from build123d import *

# Parameters (mm, degrees)
SKETCH_1_R          = 30
SKETCH_1_R_2        = 17.5
EXTRUDE_1_DEPTH     = 17.5
SKETCH_2_R          = 21
CUT_EXTRUDE_1_DEPTH = 13
CHAMFER_1_SIZE      = 1


with BuildPart() as part:
    # 草图1 → 凸台-拉伸1 (new, symmetric)
    with BuildSketch(Plane.XY):
        Circle(SKETCH_1_R)
        Circle(SKETCH_1_R_2, mode=Mode.SUBTRACT)
    extrude(amount=EXTRUDE_1_DEPTH, both=True)

    # 草图2 → 切除-拉伸1 (cut)
    with BuildSketch(Plane.XY.offset(17.5)):
        Circle(SKETCH_2_R)
    cut_extrude_1 = extrude(amount=-CUT_EXTRUDE_1_DEPTH, mode=Mode.SUBTRACT)

    # 镜向1: 切除-拉伸1 across plane
    add(cut_extrude_1.mirror(Plane.XY), mode=Mode.SUBTRACT)

    # 倒角1
    chamfer_1_edges = [part.edges().sort_by_distance(p)[0] for p in [
        (-17.5, 0, 4.5),
        (-21, 0, 17.5),
        (-21, 0, -17.5),
        (-17.5, 0, -4.5),
    ]]
    chamfer(chamfer_1_edges, length=CHAMFER_1_SIZE)


solid = part.part
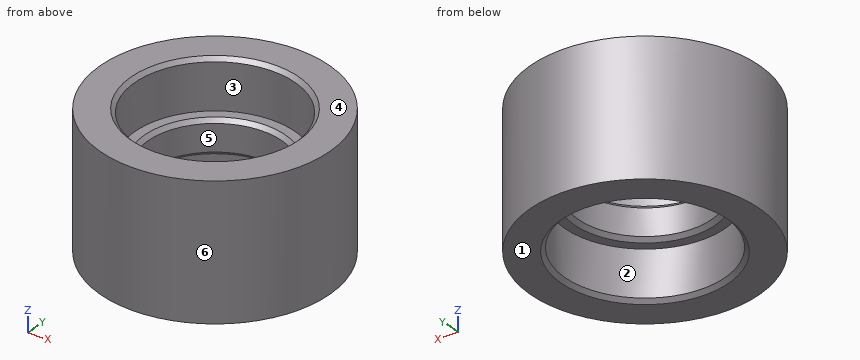
Input: part model. Units: mm. Frame: model coordinates. Face numbers are marked on the shaded views. A direction names the side the tool comes from. Give positions to 0.01 mm unless a question says otherwise; leave off trailing zeros. Order: outer loops, then holes, each group sorted by start corner. A loop starts at its lowest first (then second) coordinate and runs counter-clockwise, first axis right, second up. Notation, with made-up numbers: (0.25, 36.25) - (30.25, 36.25) arc R17 ccw to (30.25, 48.25) - close; hole circle Ø2 at (-37.75, 81.25). An arc over 180 degrees is marked (long way). Answer as a JSON object with one key per item and string values. Group by question number.
Q1. Cut plane C-C, the plane z = -7.5. Output: boundary loops of the cut face in (x, y), then the cut area to 3 significant figures.
Q2. Cut plane D-D, the plane x = 24. Output: boundary loops of the cut face in (y, z), then the cut area to 3 significant figures.
Q3. First-contact query: pin 1 Ø10 at (x, z) = (17.5, 5) entering from -Y; pin 2 Ø10 at (y, z) = (-8, 3.5) entering from +X; pin 3 Ø21 at (x, y) = (7, 1) entering from +Z; pin 4 Ø25 at (x, y) = (0, 0) entering from +Z. Flat tips, straight axial feed; report the tip coordinate or a pass-through.
Q4. Mould query, pull axis X, two halves, no side actions, for the marked faces 4, 5 and 6. Classes: pulls with the +X half, pulls with the -X half, needs draft (parallel to the pull), parting line crosses it, or undercut.
Q5. Cut plane A-A, the plane x = 0. Output: boundary loops of the cut face in (y, z), then the cut area to 3 significant figures.
Q6. Set-up query: the marked faces 1, 2 and 3. Return all of +Z, -Z, +X, -X, +Y, -Y with unobstructed straight access to the full face (end or side cutting, diameter ignored); none if empty.
Q7. Line query: probe 1 along Y at (x, z) = (0, 11); probe 2 along Y at (x, z) = (0, 1); probe 3 along Z at (x, y) = (-3, -20). Output: solid intervals per line, ascending.
Results:
{
 "1": {"outline": "circle Ø60 at (0, 0); hole circle Ø42 at (0, 0)", "area": "1,440 mm^2"},
 "2": {"outline": "(-18, -17.5) - (18, -17.5) - (18, 17.5) - (-18, 17.5) - close", "area": "1,260 mm^2"},
 "3": {"pin 1": "y = -27.27", "pin 2": "x = 29.85", "pin 3": "z = 3.57", "pin 4": "through"},
 "4": {"face 4": "needs draft", "face 5": "undercut", "face 6": "parting line crosses it"},
 "5": {"outline": "(-30, -17.5) - (-22, -17.5) - (-21, -16.5) - (-21, -4.5) - (-18.5, -4.5) - (-17.5, -3.5) - (-17.5, 3.5) - (-18.5, 4.5) - (-21, 4.5) - (-21, 16.5) - (-22, 17.5) - (-30, 17.5) - close; (17.5, -3.5) - (18.5, -4.5) - (21, -4.5) - (21, -16.5) - (22, -17.5) - (30, -17.5) - (30, 17.5) - (22, 17.5) - (21, 16.5) - (21, 4.5) - (18.5, 4.5) - (17.5, 3.5) - close", "area": "689 mm^2"},
 "6": {"face 1": "-Z, +X, -X, +Y, -Y", "face 2": "-Z", "face 3": "+Z"},
 "7": {"probe 1": "-30 to -21, 21 to 30", "probe 2": "-30 to -17.5, 17.5 to 30", "probe 3": "-4.5 to 4.5"}
}
